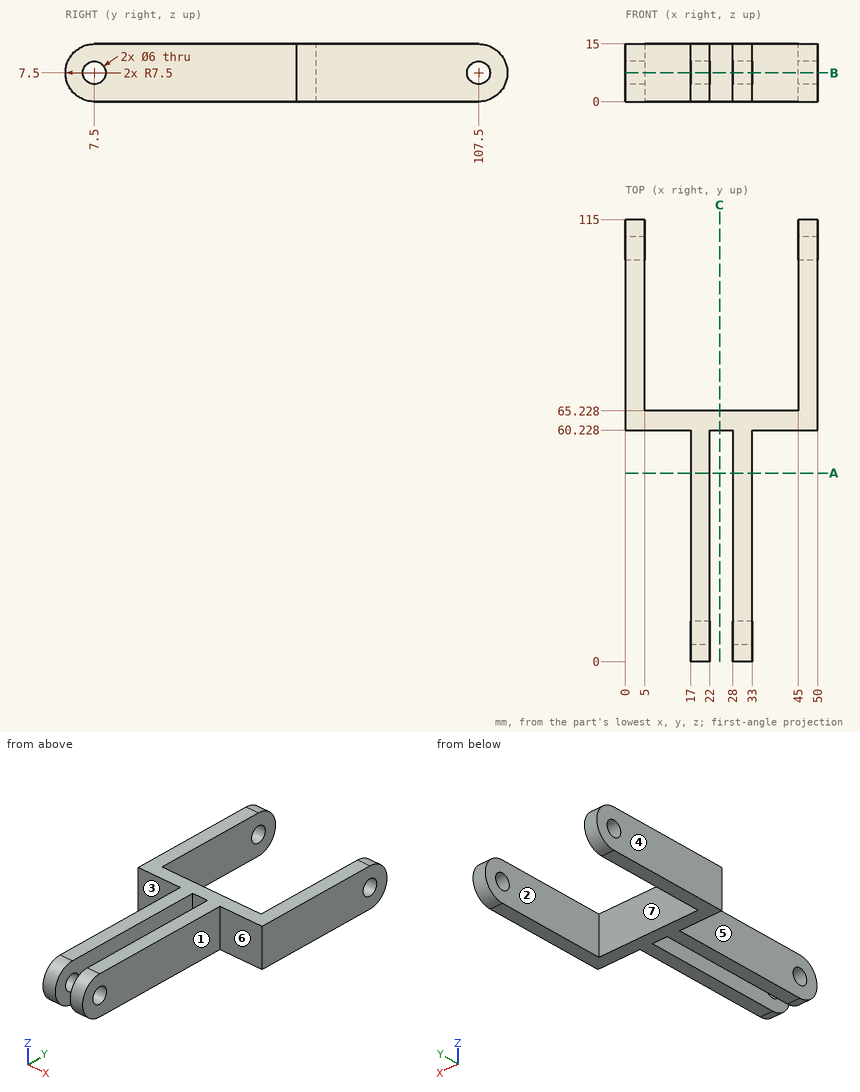
Here's the drawing with two shaded views (mm, measured from the low corner). I have some questions. A direction names the side the tool comes from. Coordinates: 2 decimals unless noted, no trailing zeros. Order: outer loops, then holes, each group sorted by start corner. A loop starts at its lowest first (then second) coordinate and runs counter-clockwise, first axis right, second up. Notation, with made-up numbers: M 73,61 L 85,61 A21 cw 85,89 Z; hole C -7.5,-34 d8. An arc over 180 degrees is marked long. Write item = value, one per line.
(1) Suppose I cut it at A-A on y = 49. Please give me the cut outline in (x, z), plus the area to 3 significant figures.
Results are:
outline = M 17,0 L 22,0 L 22,15 L 17,15 Z; M 28,0 L 33,0 L 33,15 L 28,15 Z
area = 150 mm2
(2) For the marked faces 4, 5, 6 and 7, which set-ups out of +Z, -Z, +X, -X, +Y, -Y let a thin tool reach every point of the face, with its end or its side?
Results are:
face_4 = +Z, -Z, -X, +Y, -Y
face_5 = +Z, -Z, -X, -Y
face_6 = +Z, -Z, +X, -Y
face_7 = +Z, -Z, +Y
(3) I need wall thicknesses on line 1 along X through (y, z) = (82, 10); line 2 along X through (y, z) = (21, 1.5); line 3 along Y through (x, z) = (9, 1.25). Which ranges of each line are inside material? Lowest first, please. Write a range as [from, to].
Results are:
line_1 = [0, 5], [45, 50]
line_2 = [17, 22], [28, 33]
line_3 = [60.23, 65.23]
(4) For pin 1 Ø12 at (x, y) = (34, 66) entering from -Z; pin 2 Ø1.8 at (x, z) = (26.5, 7.5) entering from -Y; pin 3 Ø8 at (x, z) = (12, 7.5) entering from +Y; pin 4 Ø1.5 at (y, z) = (29, 10) entering from +X, each with a flat end and sliding along its axis, tell me the tip position at first contact or that it passes through.
Results are:
pin_1 = 0
pin_2 = 60.23
pin_3 = 65.23
pin_4 = 33
(5) Suppose I cut it at B-B on z = 7.5. State how many separate pieces and enclosed holes the cut face has, plus the area to 3 significant figures.
Results are:
separate_pieces = 5
enclosed_holes = 0
area = 1,230 mm2
(6) If we mould it in two halves opening along X, with no side actions, what happens to the marked faces 1, 2 and 3? For each: pulls with the +X half, pulls with the -X half, needs draft (parallel to the pull), parting line crosses it, or undercut.
Results are:
face_1 = pulls with the +X half
face_2 = undercut
face_3 = needs draft
(7) Suppose I cut it at C-C on x = 24.5. Please give me the cut outline in (y, z).
Results are:
outline = M 60.23,0 L 65.23,0 L 65.23,15 L 60.23,15 Z
